```python
from build123d import *

# Parameters (mm, degrees)
SKETCH1_W           = 68
SKETCH1_H           = 225
BOSS_EXTRUDE1_DEPTH = 5
SKETCH3_R           = 5.05
CUT_EXTRUDE1_DEPTH  = 8
FILLET1_R           = 8
CUT_EXTRUDE2_DEPTH  = 118.631840928
FILLET2_R           = 10
CUT_EXTRUDE3_DEPTH  = 8
FILLET3_R           = 10
CUT_EXTRUDE4_DEPTH  = 118.631840928
FILLET4_R           = 5
FILLET5_R           = 50


with BuildPart() as part:
    # Sketch1 → Boss-Extrude1 (new body)
    with BuildSketch(Plane.XY):
        Rectangle(SKETCH1_W, SKETCH1_H)
    extrude(amount=BOSS_EXTRUDE1_DEPTH)

    # Sketch3 → Cut-Extrude1 (cut)
    with BuildSketch(Plane.XY.offset(5)):
        with Locations((22.5, -102.5)):
            Circle(SKETCH3_R)
        with Locations((13.500973464, -91.775377796)):
            Circle(SKETCH3_R)
        with Locations((4.501946929, -81.050755593)):
            Circle(SKETCH3_R)
        with Locations((-4.497079607, -70.326133389)):
            Circle(SKETCH3_R)
        with Locations((-13.496106142, -59.601511185)):
            Circle(SKETCH3_R)
        with Locations((-22.495132678, -48.876888982)):
            Circle(SKETCH3_R)
    extrude(amount=-CUT_EXTRUDE1_DEPTH, mode=Mode.SUBTRACT)

    # Fillet1
    fillet1_edges = [part.edges().sort_by_distance(p)[0] for p in [
        (34, -112.5, 2.5),
    ]]
    fillet(fillet1_edges, radius=FILLET1_R)

    # Sketch5 → Cut-Extrude2 (cut, through all)
    with BuildSketch(Plane.XY.offset(5)):
        Polygon((14.573405195, -112.5), (-34, -54.612469854), (-34, -112.5), align=None)
    extrude(amount=-CUT_EXTRUDE2_DEPTH, mode=Mode.SUBTRACT)

    # Fillet2
    fillet2_edges = [part.edges().sort_by_distance(p)[0] for p in [
        (14.573405195, -112.5, 2.5),
    ]]
    fillet(fillet2_edges, radius=FILLET2_R)

    # Sketch6 → Cut-Extrude3 (cut)
    with BuildSketch(Plane.XY.offset(5)):
        with BuildLine():
            Line((-8.5, 112.5), (-8.5, 100.171171994))
            ThreePointArc((-8.5, 100.171171994), (0, 95.835585997), (8.5, 100.171171994))
            Line((8.5, 100.171171994), (8.5, 112.5))
            ThreePointArc((8.5, 112.5), (0, 116.835585997), (-8.5, 112.5))
        make_face()
    extrude(amount=-CUT_EXTRUDE3_DEPTH, mode=Mode.SUBTRACT)

    # Fillet3
    fillet3_edges = [part.edges().sort_by_distance(p)[0] for p in [
        (-34, -54.612469854, 2.5),
    ]]
    fillet(fillet3_edges, radius=FILLET3_R)

    # Sketch7 → Cut-Extrude4 (cut, through all)
    with BuildSketch(Plane.XY.offset(5)):
        Polygon((-20, 112.5), (-34, 52.5), (-34, 112.5), align=None)
        Polygon((34, 112.5), (20, 112.5), (34, 52.5), align=None)
    extrude(amount=-CUT_EXTRUDE4_DEPTH, mode=Mode.SUBTRACT)

    # Fillet4
    fillet4_edges = [part.edges().sort_by_distance(p)[0] for p in [
        (-20, 112.5, 2.5),
        (20, 112.5, 2.5),
    ]]
    fillet(fillet4_edges, radius=FILLET4_R)

    # Fillet5
    fillet5_edges = [part.edges().sort_by_distance(p)[0] for p in [
        (-34, 52.5, 2.5),
        (34, 52.5, 2.5),
    ]]
    fillet(fillet5_edges, radius=FILLET5_R)


solid = part.part
```
CAD build for the part. Positions are in the model's coordinates, mm. A direction names the side the tool comes from. Coordinates: 2 decimals unless noted, no trailing zeros. Order: outer loops, then holes, each group sorted by start corner. A loop starts at its lowest first (then second) coordinate and runs counter-clockwise, first axis right, second up. Notation, with made-up numbers: (-33, 81) - (-3, 81) arc R29 ccw to (-3, 107) - close; hole circle Ø4 at (49, -6.75). An arc over 180 degrees is marked (long way). Use a Markdown table: item, result. Add a question column.
(1) Which spindle directions (+Z, -Z, +X, -X, +Y, -Y) get a long thin tool onto all of the face, cutting with end or side? Do faces 1 (the face through (8.5, 106, 3)), 2 (the face through (33.68, 52.38, 2.46)). Say none if no direction does.
(2) Saw through at D-D (y = 81). Give the cut face in (x, z), then the cut area to 4 significant figures.
(3) Saw through at C-C (z = 3.7). Give the cut face in (x, y).
(4) Saw through at B-B (x = 6). Give the cut face in (y, z).
(5) Flat gauge pins, fed straight in: pin 1 (2 mm diameter, centred on y = 68, z = 1.5, fed in from +X); pin 2 (8 mm diameter, centred on x = -13.5, y = -59.6, fed in from -Z); pin 3 (1.5 mm diameter, centred on y = 108.5, z = 1.5, fed in from +X). Where does each tip first touch, or does it go through?
(6) Saw through at A-A (y = -46). Give the cut face in (x, z).
(7) Drill centre lines: line 1 along Y through (x, z) = (-9, 2.7); line 2 along Y through (x, z) = (-1, 0.7); line 3 along X through (y, z) = (-59.5, 1.5). Where is each one in solid material? Low to high. Write a range as [from, to].
(8) Pull direction Y, two halves, no side cores. Call faces 3 (the face through (-26.714, 83.725, 2.535)), 4 (the face through (23, -112.5, 2)), 5 (the face through (-14.59, -64.53, 2.54)): +Y half, -Y half, draft (parallel to the pull), parting line (faces both ways), or undercut.
Solved:
| question | item | result |
|---|---|---|
| 1 | face 1 | +Z, -Z, +Y |
| 1 | face 2 | +Z, -Z, +X, +Y |
| 2 | outline | (-27.35, 0) - (27.35, 0) - (27.35, 5) - (-27.35, 5) - close |
| 2 | area | 273.5 mm² |
| 3 | outline | (-34, -50.97) arc R10 ccw to (-31.66, -57.4) - (11.58, -108.93) arc R10 ccw to (19.24, -112.5) - (26, -112.5) arc R8 ccw to (34, -104.5) - (34, 46.74) arc R50 ccw to (32.69, 58.11) - (20.9, 108.64) arc R5 ccw to (16.03, 112.5) - (8.5, 112.5) - (8.5, 100.17) arc R10.5 cw to (-8.5, 100.17) - (-8.5, 112.5) - (-16.03, 112.5) arc R5 ccw to (-20.9, 108.64) - (-32.69, 58.11) arc R50 ccw to (-34, 46.74) - close; hole circle Ø10.1 at (-22.5, -48.88); hole circle Ø10.1 at (-13.5, -59.6); hole circle Ø10.1 at (-4.5, -70.33); hole circle Ø10.1 at (4.5, -81.05); hole circle Ø10.1 at (13.5, -91.78); hole circle Ø10.1 at (22.5, -102.5) |
| 4 | outline | (-102.28, 0) - (-85.87, 0) - (-85.87, 5) - (-102.28, 5) - close; (-76.23, 0) - (97.72, 0) - (97.72, 5) - (-76.23, 5) - close |
| 5 | pin 1 | stops at x = 30.62 |
| 5 | pin 2 | passes through |
| 5 | pin 3 | stops at x = 21.11 |
| 6 | outline | (-34, 0) - (-26.65, 0) - (-26.65, 5) - (-34, 5) - close; (-18.34, 0) - (34, 0) - (34, 5) - (-18.34, 5) - close |
| 7 | line 1 | y = [-84.41, -72.61], [-68.04, -61.9], [-57.3, 112.5] |
| 7 | line 2 | y = [-93.94, -73.97], [-66.68, 95.88] |
| 7 | line 3 | x = [-29.9, -18.55], [-8.45, 34] |
| 8 | face 3 | +Y half |
| 8 | face 4 | -Y half |
| 8 | face 5 | undercut |
